```python
from build123d import *


with BuildPart() as part:
    # 草图1 → 旋转1 (revolve)
    with BuildSketch(Plane.XY):
        with BuildLine():
            Line((-36.2806, 5.587), (-36.973, 5.587))
            ThreePointArc((-36.973, 5.587), (-37.680106781, 5.879893219), (-37.973, 6.587))
            Line((-37.973, 6.587), (-37.973, 9.413))
            ThreePointArc((-37.973, 9.413), (-37.680106781, 10.120106781), (-36.973, 10.413))
            Line((-36.973, 10.413), (-36.2806, 10.413))
            ThreePointArc((-36.2806, 10.413), (-35.573493219, 10.120106781), (-35.2806, 9.413))
            Line((-35.2806, 9.413), (-35.2806, 6.587))
            ThreePointArc((-35.2806, 6.587), (-35.573493219, 5.879893219), (-36.2806, 5.587))
        make_face()
    revolve(axis=Axis((0, 27, 0), (0, -1, 0)))


solid = part.part
```
Here's how the part is built. I have some questions about the finished solid (model axes, mm). Round coordinates to 2 decimals unless told otherwise and drop trailing zeros. Order: outer loops, then holes, each group sorted by start corner. A loop starts at its lowest first (then second) coordinate and runs counter-clockwise, first axis right, second up. Notation, with made-up numbers: M -2,24.25 L 43,24.25 A24 cw 43,51.25 Z; hole C 13,10 d7. An arc over 180 degrees is marked long. One line per question, with ' | ' between items.
1) I want a section at C-C, the plane y = 8.35. Write out the boundary of the cut face in (x, z).
Working result:
outline: C 0,0 d75.95; hole C 0,0 d70.56
2) I want a section at A-A, the plane z = 0. Write out the boundary of the cut face in (x, y).
Working result:
outline: M -37.97,6.59 A1 ccw -36.97,5.59 L -36.28,5.59 A1 ccw -35.28,6.59 L -35.28,9.41 A1 ccw -36.28,10.41 L -36.97,10.41 A1 ccw -37.97,9.41 Z; M 35.28,6.59 A1 ccw 36.28,5.59 L 36.97,5.59 A1 ccw 37.97,6.59 L 37.97,9.41 A1 ccw 36.97,10.41 L 36.28,10.41 A1 ccw 35.28,9.41 Z
3) I want a section at B-B, the plane x = 0. Write out the boundary of the cut face in (y, z).
Working result:
outline: M 5.59,-36.97 A1 ccw 6.59,-37.97 L 9.41,-37.97 A1 ccw 10.41,-36.97 L 10.41,-36.28 A1 ccw 9.41,-35.28 L 6.59,-35.28 A1 ccw 5.59,-36.28 Z; M 5.59,36.28 A1 ccw 6.59,35.28 L 9.41,35.28 A1 ccw 10.41,36.28 L 10.41,36.97 A1 ccw 9.41,37.97 L 6.59,37.97 A1 ccw 5.59,36.97 Z
4) I need wall thicknesses on line 1 along X through (y, z) = (7.35, 0); line 2 along X through (y, z) = (6.55, -28.5). Which ranges of each line are inside material? Lowest first, please.
Working result:
line 1: -37.97 to -35.28, 35.28 to 37.97 | line 2: -25.09 to -20.8, 20.8 to 25.09
5) If we mould it in two halves opening along Z, with no side actions, what happens to faces 1 (the face through (27.997, 7.98, 21.468)), 2 (the face through (-24.5, 10.413, 27.2)), 3 (the face through (-36.22, 8.02, -11.41))? For each: +Z half, -Z half, draft (parallel to the pull), parting line (faces both ways), or undercut.
Working result:
face 1: undercut | face 2: draft | face 3: parting line
6) For pin 1 Ø2 at (x, y) = (15, 7) entering from +Z; pin 2 Ø1.5 at (y, z) = (6.5, 25) entering from +X; pin 3 Ø6 at (x, z) = (-27.5, -16.5) entering from -Y, each with a flat end and sliding along its axis, tell me the tip position at first contact or that it passes through.
Working result:
pin 1: z = 35.3 | pin 2: x = 29.22 | pin 3: through
